Source: CAD feature listing. Evaluate the final solid. Frame: model axes, mm. Face numbers are marked on the shaded views. A direction names the side the tool comes from. Coordinates: 2 decimals unless noted, no trailing zeros. Loops run counter-clockwise (first coordinate to the right, second up) from the corner with the lowest first, then second, coordinate; pieces in that order, holes last. Notation, with made-up numbers: M 31.5,35 L 39.5,35 A14 ccw 39.5,44 Z; hole C 66,83.5 d10. An arc over 180 degrees is marked long. Write each question's results on one line, items separated by ' | '. Start each with the question number.
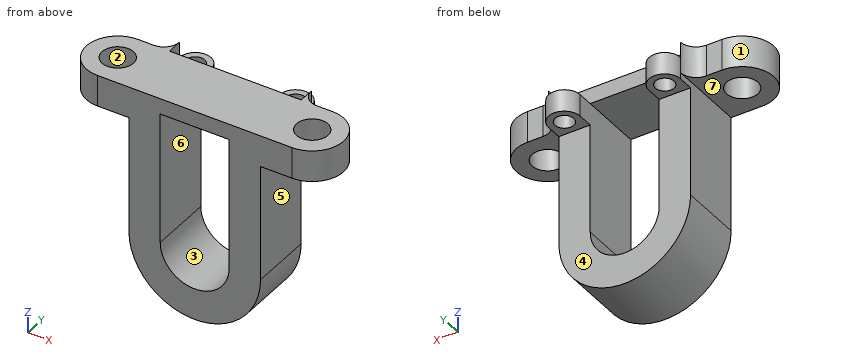
from build123d import *

# Parameters (mm, degrees)
BASE_PLATE_SKETCH_W    = 42
BASE_PLATE_SKETCH_H    = 20
BASE_PLATE_DEPTH       = 5
CURVED_LOOP_BOSS_DEPTH = 20
LOOP_SLOT_CUT_DEPTH    = 79.31347266
LUG_SKETCH_R           = 3
LUG_BOSS_DEPTH         = 7
PIN_EYE_SKETCH_R       = 5
PIN_EYE_BOSS_DEPTH     = 5


with BuildPart() as part:
    # Base Plate Sketch → Base Plate (new body)
    with BuildSketch(Plane.XY):
        with Locations((21, 10)):
            Rectangle(BASE_PLATE_SKETCH_W, BASE_PLATE_SKETCH_H)
    extrude(amount=BASE_PLATE_DEPTH)

    # Curved Loop Sketch → Curved Loop Boss (add, through all)
    with BuildSketch(Plane(origin=(0, 20, 0), x_dir=(1, 0, 0), z_dir=(0, 1, 0))):
        with BuildLine():
            Line((0, 42), (0, 0))
            Line((0, 0), (42, 0))
            Line((42, 0), (42, 42))
            ThreePointArc((42, 42), (21, 63), (0, 42))
        make_face()
    extrude(amount=-CURVED_LOOP_BOSS_DEPTH)

    # Loop Slot Sketch → Loop Slot Cut (cut, through all)
    with BuildSketch(Plane(origin=(0, 20, 0), x_dir=(1, 0, 0), z_dir=(0, 1, 0))):
        with BuildLine():
            Line((10, 42), (10, 0))
            Line((10, 0), (32, 0))
            Line((32, 0), (32, 42))
            ThreePointArc((32, 42), (21, 53), (10, 42))
        make_face()
    extrude(amount=-LOOP_SLOT_CUT_DEPTH, mode=Mode.SUBTRACT)

    # Lug Sketch → Lug Boss (add)
    with BuildSketch(Plane.XY):
        with BuildLine():
            Line((0, 25), (0, 20))
            Line((0, 20), (10, 20))
            Line((10, 20), (10, 25))
            ThreePointArc((10, 25), (5, 30), (0, 25))
        make_face()
        with Locations((5, 25)):
            Circle(LUG_SKETCH_R, mode=Mode.SUBTRACT)
    lug_boss = extrude(amount=-LUG_BOSS_DEPTH)

    # Lug Mirror: Lug Boss across plane
    add(lug_boss.mirror(Plane(origin=(21, 0, 0), x_dir=(0, 0, 1), z_dir=(1, 0, 0))))

    # Pin Eye Sketch → Pin Eye Boss (add, symmetric)
    with BuildSketch(Plane.XY):
        with BuildLine():
            Line((-10, 20), (-5, 20))
            ThreePointArc((-5, 20), (-1.464466094, 21.464466094), (0, 25))
            Line((0, 25), (0, 20))
            Line((0, 20), (0, 0))
            Line((0, 0), (-10, 0))
            ThreePointArc((-10, 0), (-20, 10), (-10, 20))
        make_face()
        with Locations((-10, 10)):
            Circle(PIN_EYE_SKETCH_R, mode=Mode.SUBTRACT)
    pin_eye_boss = extrude(amount=PIN_EYE_BOSS_DEPTH, both=True)

    # Pin Eye Mirror: Pin Eye Boss across plane
    add(pin_eye_boss.mirror(Plane(origin=(21, 0, 0), x_dir=(0, 0, 1), z_dir=(1, 0, 0))))


solid = part.part
Item 1: Line query: probe 1 along X at (y, z) = (6.5, -25.5); probe 2 along Y at (x, z) = (5, -2); probe 3 along Y at (x, z) = (-10, 0). Output: solid intervals per line, ascending.
Item 2: Access query for the marked faces 4, 5, 6 and 7. Directions: +Z, -Z, +X, -X, +Y, -Y. A direction counts if a zero-diameter tool reaches every point of the face in a straight line with its end or side. Return the directions, or none.
Item 3: Mould query, pull axis Y, two halves, no side actions, for the marked faces 1, 2 and 3. Classes: +Y half, -Y half, draft (parallel to the pull), parting line (faces both ways), or undercut.
Item 4: Cut plane B-B (y = 10). Output: boundary loops of the cut face in (x, z).
Item 5: Cut plane D-D (x = 36.5). Output: boundary loops of the cut face in (y, z), then the cut area to 3 significant figures.
Item 6: Cut plane C-C (x = 21). Output: boundary loops of the cut face in (y, z).
Item 7: First-contact query: pin 1 Ø5 at (x, y) = (36, 25.5) entering from -Z; pin 2 Ø1.5 at (x, z) = (-7.5, -2) entering from +Y; pin 3 Ø8 at (x, y) = (38, 26.5) entering from +Z; pin 4 Ø6 at (x, y) = (48.5, 10) entering from +Z. Flat tips, straight axial feed; report the tip coordinate or a pass-through.
Item 8: Cut plane A-A (z = -38). Output: boundary loops of the cut face in (x, y).
Response values:
1) probe 1: x = 0 to 10, 32 to 42 | probe 2: y = 0 to 22, 28 to 30 | probe 3: y = 0 to 5, 15 to 20
2) face 4: -Z, +X, -X, +Y | face 5: -Z, +X, +Y, -Y | face 6: +Y, -Y | face 7: -Z, -X, +Y, -Y
3) face 1: parting line | face 2: undercut | face 3: draft
4) outline: M -20,-5 L -15,-5 L -15,5 L -20,5 Z; M -5,-5 L 0,-5 L 0,-42 A21 ccw 42,-42 L 42,-5 L 47,-5 L 47,5 L -5,5 Z; M 57,-5 L 62,-5 L 62,5 L 57,5 Z; hole M 10,-42 A11 ccw 32,-42 L 32,0 L 10,0 Z
5) outline: M 0,-56.17 L 20,-56.17 L 20,-7 L 22.04,-7 L 22.04,0 L 20,0 L 20,5 L 0,5 Z; M 27.96,-7 L 29.97,-7 L 29.97,0 L 27.96,0 Z | area: 1,250 mm2
6) outline: M 0,-63 L 20,-63 L 20,-53 L 0,-53 Z; M 0,0 L 20,0 L 20,5 L 0,5 Z
7) pin 1: stops at z = -7 | pin 2: stops at y = 20 | pin 3: stops at z = 0 | pin 4: stops at z = 5
8) outline: M 0,0 L 10,0 L 10,20 L 0,20 Z; M 32,0 L 42,0 L 42,20 L 32,20 Z
